```python
from build123d import *

# Parameters (mm, degrees)
SKETCH_1_W        = 1480
SKETCH_1_H        = 210
SKETCH_1_W_2      = 1470
SKETCH_1_H_2      = 200
EXTRUDE_1_DEPTH   = 70
SKETCH_2_W        = 5
SKETCH_2_H        = 210
EXTRUDE_1_2_DEPTH = 1470


with BuildPart() as part:
    # 草图1 → Extrude 1 (new body)
    with BuildSketch(Plane.XY):
        Rectangle(SKETCH_1_W, SKETCH_1_H)
        Rectangle(SKETCH_1_W_2, SKETCH_1_H_2, mode=Mode.SUBTRACT)
    extrude(amount=EXTRUDE_1_DEPTH)

    # 草图2 → Extrude 1 2 (add)
    with BuildSketch(Plane.ZY.offset(-735)):
        with Locations((2.5, 0)):
            Rectangle(SKETCH_2_W, SKETCH_2_H)
    extrude(amount=EXTRUDE_1_2_DEPTH)


solid = part.part
```
The model under review builds one solid part; all positions refer to its coordinate system, in mm. A direction names the side the tool comes from. Round coordinates to 2 decimals unless told otherwise and drop trailing zeros. Loops run counter-clockwise (first coordinate to the right, second up) from the corner with the lowest first, then second, coordinate; pieces in that order, holes last.
Item 1: Mouldability with a two-part tool opening along X and no side actions: class faces 3 (the face through (10, -105, 35)), 4 (the face through (-740, -1, 35)), 5 (the face through (735, -1, 37)) as released by +X, released by -X, zero draft, split by the parting line, or undercut.
Determined:
face 3: zero draft
face 4: released by -X
face 5: undercut
Item 2: For faces 1 (the face through (-10, 105, 35)), 2 (the face through (-10, -100, 37)), list the 3-axis set-ups (+Z, -Z, +X, -X, +Y, -Y) from which the entire face can be reached by the end or side of a thin tool; tool diameter is ignored.
Determined:
face 1: +Z, -Z, +X, -X, +Y
face 2: +Z
Item 3: Take a section at B-B (y = -10.5). Write out the cut boundary in (x, z), then the cut area to 3 significant figures.
Determined:
outline: (-740, 0) - (740, 0) - (740, 70) - (735, 70) - (735, 5) - (-735, 5) - (-735, 70) - (-740, 70) - close
area: 8,050 mm2
Item 4: Clearance check with a flat-ended pin moving along its axis: pin 1 Ø5 at (x, y) = (402.5, -15) entering from -Z. State where the tip first meets the part, or that it passes through.
Determined:
pin 1: stops at z = 0
Item 5: Take a section at C-C (x = 139.5). Write out the cut boundary in (y, z), then the cut area to 3 significant figures.
Determined:
outline: (-105, 0) - (105, 0) - (105, 70) - (100, 70) - (100, 5) - (-100, 5) - (-100, 70) - (-105, 70) - close
area: 1,700 mm2
Item 6: For line 1 (Y direction, x = -74.5, z = 17); line 2 (X direction, y = 2, z = 12.5); line 3 (Z direction, x = -521.5, y = -27), list the stretches that pass through material, from the lowest coordinate up.
Determined:
line 1: y = -105 to -100, 100 to 105
line 2: x = -740 to -735, 735 to 740
line 3: z = 0 to 5
Item 7: Take a section at A-A (z = 24). Write out the cut boundary in (x, y), then the cut area to 3 significant figures.
Determined:
outline: (-740, -105) - (740, -105) - (740, 105) - (-740, 105) - close; hole (-735, -100) - (735, -100) - (735, 100) - (-735, 100) - close
area: 16,800 mm2
